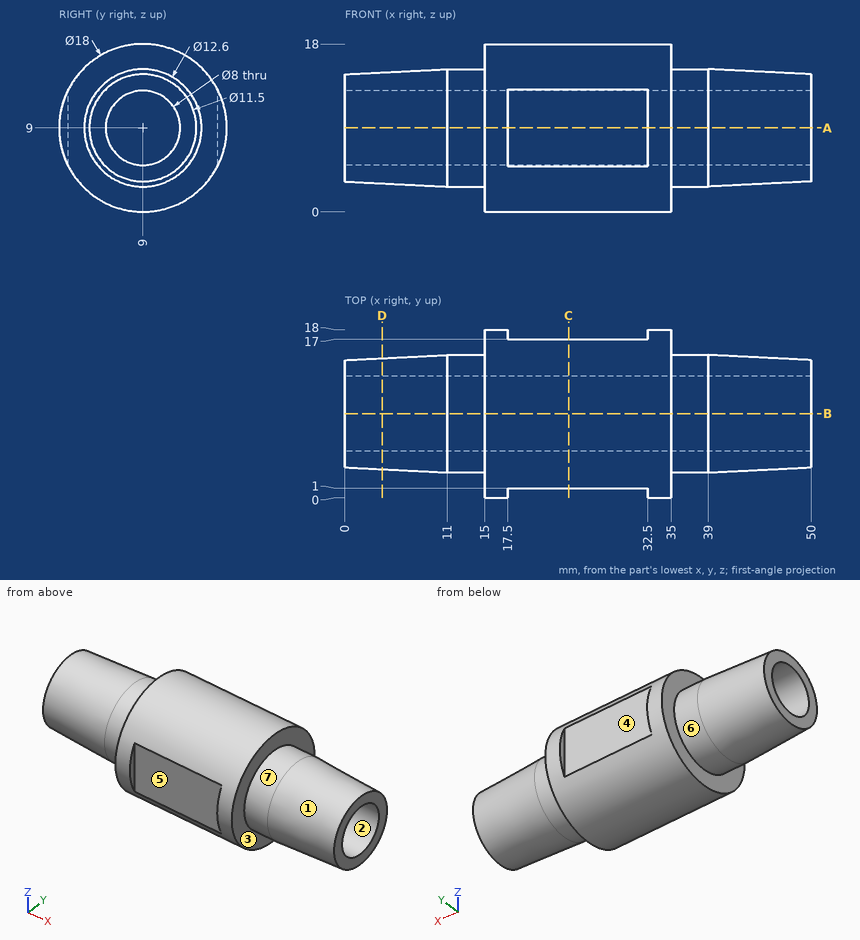
Can you work these out from the drawing? Everything is in mm from the part's minimum corner. A direction names the side the tool comes from. Coordinates: 2 decimals unless noted, no trailing zeros. Write each loop counter-clockwise with the first axis right and the second up, starting at its lowest first coordinate (ties: lowest second). Pieces come first, ordered by that corner, then holes. Notation, with made-up numbers: (47, -21) -> (54, -21) arc R14 ccw to (54, -14) -> close; hole circle Ø9 at (-29, 0). An arc over 180 degrees is marked (long way). Return JSON: item names as keys, results as strings.
(1) Imagine slicing it at B-B, the plane y = 9. Please give me the cut outline in (x, z), then the cut area to 3 significant figures.
Numbers:
{"outline": "(0, 3.25) -> (11, 2.7) -> (15, 2.7) -> (15, 0) -> (35, 0) -> (35, 2.7) -> (39, 2.7) -> (50, 3.25) -> (50, 5) -> (0, 5) -> close; (0, 13) -> (50, 13) -> (50, 14.75) -> (39, 15.3) -> (35, 15.3) -> (35, 18) -> (15, 18) -> (15, 15.3) -> (11, 15.3) -> (0, 14.75) -> close", "area": "326 mm2"}
(2) Imagine slicing it at C-C, the plane x = 24. Please give me the cut outline in (y, z), then the cut area to 3 significant figures.
Numbers:
{"outline": "(1, 4.88) arc R9 ccw to (17, 4.88) -> (17, 13.12) arc R9 ccw to (1, 13.12) -> close; hole circle Ø8 at (9, 9)", "area": "193 mm2"}
(3) We'd pull the mould along Y, two halves only. Please class the marked faces 1, 2, 3 and 4: +Y half, -Y half, draft (parallel to the pull), parting line (faces both ways), or undercut.
Numbers:
{"face 1": "parting line", "face 2": "undercut", "face 3": "draft", "face 4": "+Y half"}
(4) Imagine slicing it at A-A, the plane z = 9. Please give me the cut outline in (x, y).
Numbers:
{"outline": "(0, 3.25) -> (11, 2.7) -> (15, 2.7) -> (15, 0) -> (17.5, 0) -> (17.5, 1) -> (32.5, 1) -> (32.5, 0) -> (35, 0) -> (35, 2.7) -> (39, 2.7) -> (50, 3.25) -> (50, 5) -> (0, 5) -> close; (0, 13) -> (50, 13) -> (50, 14.75) -> (39, 15.3) -> (35, 15.3) -> (35, 18) -> (32.5, 18) -> (32.5, 17) -> (17.5, 17) -> (17.5, 18) -> (15, 18) -> (15, 15.3) -> (11, 15.3) -> (0, 14.75) -> close"}
(5) Which directions (+Z, -Z, +X, -X, +Y, -Y) give clear straight access to the entire face, cutting with the end or side of a thin tool? Please do the marked faces 5, 6 and 7.
Numbers:
{"face 5": "+Z, -Z, -Y", "face 6": "-X", "face 7": "+X"}
(6) Imagine slicing it at D-D, the plane x = 4. Please give me the cut outline in (y, z), then the cut area to 3 significant figures.
Numbers:
{"outline": "circle Ø11.9 at (9, 9); hole circle Ø8 at (9, 9)", "area": "61.0 mm2"}
(7) I need wall thicknesses on L1, parallel to Y at x = 23.5, z = 9; L2, parallel to Z at x = 25, y = 9; L3, parallel to X at y = 1.25, z = 7.5. Which ranges of each line are inside material? Lowest first, please.
Numbers:
{"L1": "y = 1 to 5, 13 to 17", "L2": "z = 0 to 5, 13 to 18", "L3": "x = 15 to 35"}
(8) I'm going to push flat-ended pins straight in: pin 1 (0.8 mm diameter, centred on y = 17.5, z = 9.5, fed in from -X); pin 2 (2 mm diameter, centred on x = 21, z = 16, fed in from +Y); pin 3 (6.5 mm diameter, centred on x = 22.5, z = 10.5, fed in from -Y). Where does each tip first touch, or does it pass through?
Numbers:
{"pin 1": "stops at x = 15", "pin 2": "stops at y = 15.71", "pin 3": "stops at y = 1"}
